Geometry check sheet. Reference: the model listing, model coordinates, mm. Face numbers are marked on the shaded views. A direction names the side the tool comes from. Give positions to 0.01 mm unless a question says otherwise; leave off trailing zeros. Write each loop counter-clockwise with the first axis right and the second up, starting at its lowest first coordinate (ties: lowest second). Pieces come first, ordered by that corner, then holes. Notation, with made-up numbers: (57.25, 51.5) -> (69.25, 51.5) arc R25 cw to (69.25, 78.5) -> close; hole circle Ø3 at (-34.75, -26). An arc over 180 degrees is marked (long way). Write item = value, one per line. Start each with the question number.
1. Thickness scan on line 1 along Z through (x, y) = (80, 10); line 2 along Z through (x, y) = (20, 4); line 3 along X through (y, z) = (10.25, -17). Record the ranges inside material, lowest first.
2. Cross-section at A-A, the plane x = 46. Record the cut outline in (y, z), plus the area to 3 significant figures.
3. Cross-section at B-B, the plane z = -8. Record the cut outline in (x, y).
4. Depth check by flat-ended pin: P1, Ø3.5, axis at x = 20, z = -8, coming from the +Y side; P2, Ø13.5, axis at x = 42.5, z = 4, coming from the +Y side; P3, Ø3, axis at x = 80.5, z = -14.5, coming from the -Y side. Enter the tip coordinate at first touch or a pass-through.
5. Cross-section at D-D, the plane y = 41. Record the cut outline in (x, z).
6. Set-up check for the marked faces 1 and 2: record each of +Z, -Z, +X, -X, +Y, -Y from which the full face is reachable in a straight line by a thin tool's end or side.
7. Cross-section at C-C, the plane x = 80. Record the cut outline in (y, z).
```python
from build123d import *

# Parameters (mm, degrees)
BOSS_EXTRUDE1_DEPTH                                  = 22.5
HOLE_SIZE_PER_SOCKET_HEAD_CAP_SCREW_TYPE_D           = 5.5
HOLE_SIZE_PER_SOCKET_HEAD_CAP_SCREW_TYPE_CBORE_D     = 10
HOLE_SIZE_PER_SOCKET_HEAD_CAP_SCREW_TYPE_CBORE_DEPTH = 5.7
F_4_5_4_5_DIAMETER_HOLE1_D                           = 4.5
M4_TAPPED_HOLE1_D                                    = 3.3
M4_TAPPED_HOLE1_DEPTH                                = 10.1
M4_TAPPED_HOLE1_TIP                                  = 0.991420021
M6_TAPPED_HOLE1_D                                    = 5
M6_TAPPED_HOLE1_DEPTH                                = 15
M6_TAPPED_HOLE1_TIP                                  = 1.502151548
F_4_0_4_DIAMETER_HOLE1_D                             = 4
F_4_0_4_DIAMETER_HOLE1_DEPTH                         = 15
F_4_0_4_DIAMETER_HOLE1_TIP                           = 1.201721238
F_4_0_4_DIAMETER_HOLE2_D                             = 4
F_4_0_4_DIAMETER_HOLE2_DEPTH                         = 17
F_4_0_4_DIAMETER_HOLE2_TIP                           = 1.201721238
CHAMFER1_SIZE                                        = 2
CHAMFER2_SIZE                                        = 1
FILLET1_R                                            = 2


with BuildPart() as part:
    # Sketch1 → Boss-Extrude1 (new, symmetric)
    with BuildSketch(Plane.XY):
        Polygon((0, 0), (0, 60), (12, 60), (12, 17), (105, 17), (105, 0), align=None)
    extrude(amount=BOSS_EXTRUDE1_DEPTH, both=True)

    # Hole size per socket head cap screw type 1 (through all)
    with Locations(Plane(origin=(0, 0, 0), x_dir=(-1, 0, 0), z_dir=(0, -1, 0))):
        with Locations((-80, -7), (-56, -7), (-56, 17), (-80, 17)):
            CounterBoreHole(HOLE_SIZE_PER_SOCKET_HEAD_CAP_SCREW_TYPE_D / 2, HOLE_SIZE_PER_SOCKET_HEAD_CAP_SCREW_TYPE_CBORE_D / 2, HOLE_SIZE_PER_SOCKET_HEAD_CAP_SCREW_TYPE_CBORE_DEPTH)

    # Ø4.5 (4.5) Diameter Hole1 (through all)
    with Locations(Plane(origin=(0, 17, 0), x_dir=(1, 0, 0), z_dir=(0, 1, 0))):
        with Locations((20, 8), (46, 8), (20, -18), (46, -18)):
            Hole(F_4_5_4_5_DIAMETER_HOLE1_D / 2)

    # M4 Tapped Hole1
    with Locations(Plane(origin=(105, 0, 0), x_dir=(0, 0, -1), z_dir=(1, 0, 0))):
        with Locations((-1, 8), (11, 8)):
            Hole(M4_TAPPED_HOLE1_D / 2, depth=M4_TAPPED_HOLE1_DEPTH)
            with Locations((0, 0, -(M4_TAPPED_HOLE1_DEPTH + M4_TAPPED_HOLE1_TIP / 2))):  # 118° drill point
                Cone(0, M4_TAPPED_HOLE1_D / 2, M4_TAPPED_HOLE1_TIP, mode=Mode.SUBTRACT)

    # M6 Tapped Hole1
    with Locations(Plane.ZY):
        with Locations((-12.5, 50), (12.5, 50), (-12.5, 10), (12.5, 10)):
            Hole(M6_TAPPED_HOLE1_D / 2, depth=M6_TAPPED_HOLE1_DEPTH)
            with Locations((0, 0, -(M6_TAPPED_HOLE1_DEPTH + M6_TAPPED_HOLE1_TIP / 2))):  # 118° drill point
                Cone(0, M6_TAPPED_HOLE1_D / 2, M6_TAPPED_HOLE1_TIP, mode=Mode.SUBTRACT)

    # Ø4.0 (4) Diameter Hole1
    with Locations(Plane.ZY):
        with Locations((-12.5, 30), (12.5, 30)):
            Hole(F_4_0_4_DIAMETER_HOLE1_D / 2, depth=F_4_0_4_DIAMETER_HOLE1_DEPTH)
            with Locations((0, 0, -(F_4_0_4_DIAMETER_HOLE1_DEPTH + F_4_0_4_DIAMETER_HOLE1_TIP / 2))):  # 118° drill point
                Cone(0, F_4_0_4_DIAMETER_HOLE1_D / 2, F_4_0_4_DIAMETER_HOLE1_TIP, mode=Mode.SUBTRACT)

    # Ø4.0 (4) Diameter Hole2
    with Locations(Plane(origin=(0, 0, 0), x_dir=(-1, 0, 0), z_dir=(0, -1, 0))):
        with Locations((-20, 15.5), (-46, 15.5)):
            Hole(F_4_0_4_DIAMETER_HOLE2_D / 2, depth=F_4_0_4_DIAMETER_HOLE2_DEPTH)
            with Locations((0, 0, -(F_4_0_4_DIAMETER_HOLE2_DEPTH + F_4_0_4_DIAMETER_HOLE2_TIP / 2))):  # 118° drill point
                Cone(0, F_4_0_4_DIAMETER_HOLE2_D / 2, F_4_0_4_DIAMETER_HOLE2_TIP, mode=Mode.SUBTRACT)

    # Chamfer1
    chamfer1_edges = [part.edges().sort_by_distance(p)[0] for p in [
        (6, 60, 22.5),
        (6, 60, -22.5),
        (105, 8.5, 22.5),
        (105, 8.5, -22.5),
    ]]
    chamfer(chamfer1_edges, length=CHAMFER1_SIZE)

    # Chamfer2
    chamfer2_edges = [part.edges().sort_by_distance(p)[0] for p in [
        (0, 0, 0),
    ]]
    chamfer(chamfer2_edges, length=CHAMFER2_SIZE)

    # Fillet1
    fillet1_edges = [part.edges().sort_by_distance(p)[0] for p in [
        (12, 17, 0),
    ]]
    fillet(fillet1_edges, radius=FILLET1_R)


solid = part.part
```
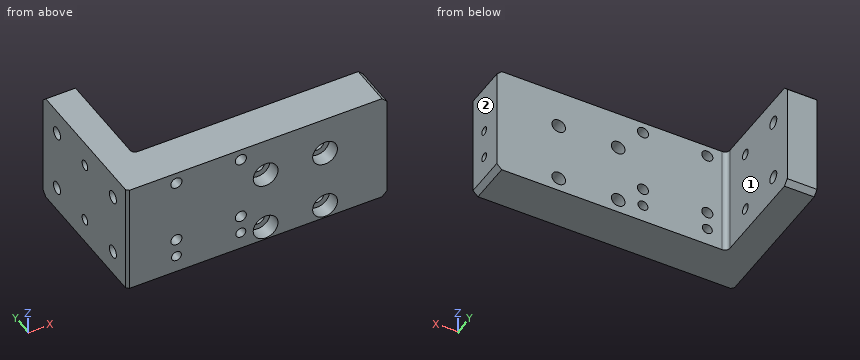
Answers:
q1.line_1 = -22.5 to -19.75, -14.25 to 4.25, 9.75 to 22.5
q1.line_2 = -22.5 to -17.5, -13.5 to -10.25, -5.75 to 15.75, 20.25 to 22.5
q1.line_3 = 0 to 18.68, 21.32 to 44.68, 47.32 to 53.25, 58.75 to 77.25, 82.75 to 105
q2.outline = (0, -22.5) -> (17, -22.5) -> (17, -17.5) -> (0, -17.5) -> close; (0, -13.5) -> (17, -13.5) -> (17, -10.25) -> (0, -10.25) -> close; (0, -5.75) -> (17, -5.75) -> (17, 15.75) -> (0, 15.75) -> close; (0, 20.25) -> (17, 20.25) -> (17, 22.5) -> (0, 22.5) -> close
q2.area = 544 mm^2
q3.outline = (0, 1) -> (1, 0) -> (17.75, 0) -> (17.75, 17) -> (14, 17) arc R2 cw to (12, 19) -> (12, 60) -> (0, 60) -> close; (22.25, 0) -> (43.75, 0) -> (43.75, 17) -> (22.25, 17) -> close; (48.25, 0) -> (105, 0) -> (105, 17) -> (48.25, 17) -> close
q4.P1 = through
q4.P2 = 17
q4.P3 = 5.7
q5.outline = (0, -22.5) -> (12, -22.5) -> (12, 22.5) -> (0, 22.5) -> close
q6.face_1 = +Z, -Z, +X, +Y
q6.face_2 = +Z, -Z, +X, +Y, -Y
q7.outline = (0, -22.5) -> (17, -22.5) -> (17, -19.75) -> (5.7, -19.75) -> (5.7, -22) -> (0, -22) -> close; (0, -12) -> (5.7, -12) -> (5.7, -14.25) -> (17, -14.25) -> (17, 4.25) -> (5.7, 4.25) -> (5.7, 2) -> (0, 2) -> close; (0, 12) -> (5.7, 12) -> (5.7, 9.75) -> (17, 9.75) -> (17, 22.5) -> (0, 22.5) -> close
